Could you check a few things on this drawing? It's one solid part, dimensions in mm from its lowest x, y, z. A direction names the side the tool comes from. Round coordinates to 2 decimals unless told otherwise and drop trailing zeros. Loops run counter-clockwise (first coordinate to the right, second up) from the corner with the lowest first, then second, coordinate; pieces in that order, holes last. Notation, with made-up numbers: (36.25, -10) -> (59.25, -10) arc R26 ccw to (59.25, 26) -> close; hole circle Ø10 at (-3, 45). An arc over 180 degrees is marked (long way). Write each question's results on one line, items separated by ' | '.
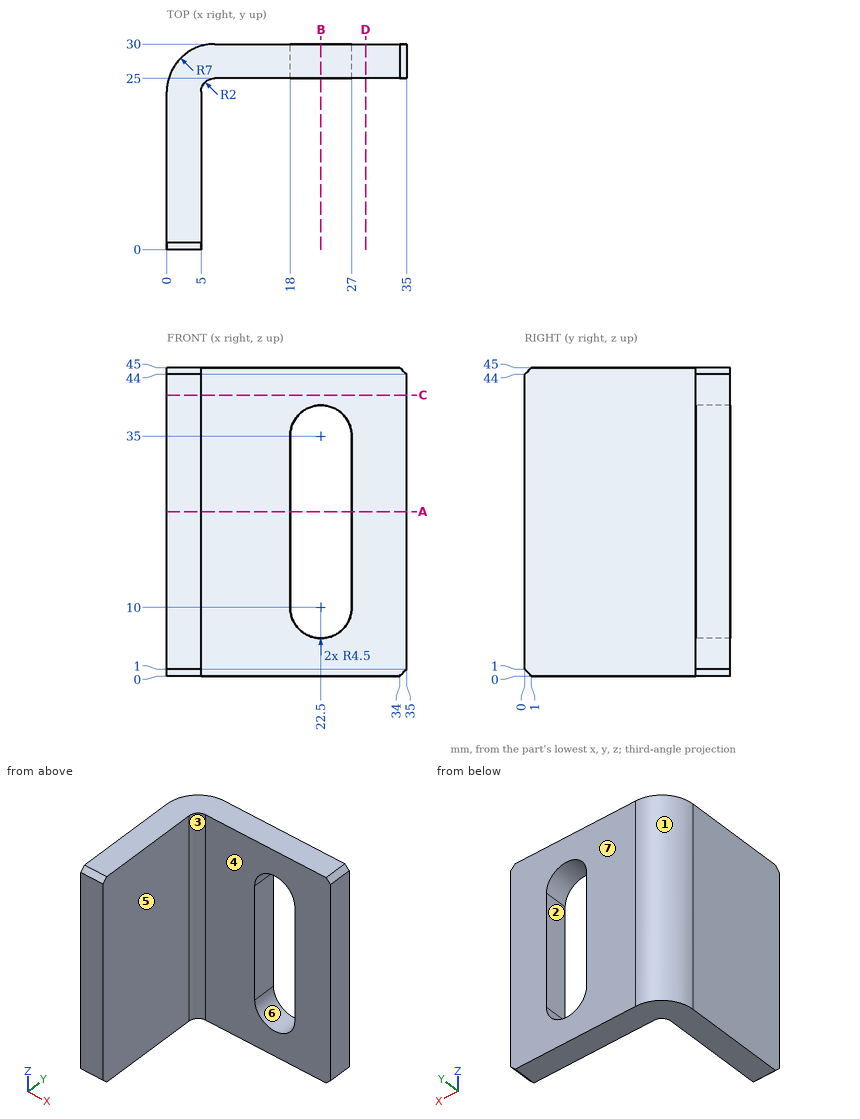
1) I'm going to push flat-ended pins straight in: pin 1 (8.5 mm diameter, centred on x = 24, z = 29.5, fed in from -Y); pin 2 (11.5 mm diameter, centred on y = 15, z = 14, fed in from +X); pin 3 (5.5 mm diameter, centred on y = 26.5, z = 18, fed in from -X). Where does each tip first touch, or does it pass through?
Model answer:
pin 1: stops at y = 25 | pin 2: stops at x = 5 | pin 3: stops at x = 0.04
2) I want a section at C-C, the plane z = 41. Write out the boundary of the cut face in (x, y).
Model answer:
outline: (0, 0) -> (5, 0) -> (5, 23) arc R2 cw to (7, 25) -> (35, 25) -> (35, 30) -> (7, 30) arc R7 ccw to (0, 23) -> close
3) I want a section at D-D, the plane x = 29. Write out the boundary of the cut face in (y, z), plus the area to 3 significant figures.
Model answer:
outline: (25, 0) -> (30, 0) -> (30, 45) -> (25, 45) -> close | area: 225 mm2
4) I need wall thicknesses on line 1 (Y direction, x = 10.5, z = 16.5); line 2 (X direction, y = 16, z = 25); line 3 (X direction, y = 25.25, z = 16.5). Which ranges of each line are inside material? Lowest first, please.
Model answer:
line 1: y = 25 to 30 | line 2: x = 0 to 5 | line 3: x = 0.37 to 18, 27 to 35
5) If we mould it in two halves opening along X, with no side actions, what happens to the marked faces 1, 2, 3 and 4? For each: released by +X, released by -X, zero draft, split by the parting line, or undercut.
Model answer:
face 1: released by -X | face 2: undercut | face 3: released by +X | face 4: zero draft
6) I want a section at A-A, the plane z = 24. Write out the boundary of the cut face in (x, y), plus the area to 3 significant figures.
Model answer:
outline: (0, 0) -> (5, 0) -> (5, 23) arc R2 cw to (7, 25) -> (18, 25) -> (18, 30) -> (7, 30) arc R7 ccw to (0, 23) -> close; (27, 25) -> (35, 25) -> (35, 30) -> (27, 30) -> close | area: 245 mm2
7) I want a section at B-B, the plane x = 22.5. Write out the boundary of the cut face in (y, z), plus the area to 3 significant figures.
Model answer:
outline: (25, 0) -> (30, 0) -> (30, 5.5) -> (25, 5.5) -> close; (25, 39.5) -> (30, 39.5) -> (30, 45) -> (25, 45) -> close | area: 55.0 mm2
8) For the marked faces 5, 6 and 7, which set-ups out of +Z, -Z, +X, -X, +Y, -Y let a thin tool reach every point of the face, with its end or its side?
Model answer:
face 5: +Z, -Z, +X, -Y | face 6: +Y, -Y | face 7: +Z, -Z, +X, -X, +Y
